```python
from build123d import *

# Parameters (mm, degrees)
SKETCH1_R           = 10.75
SKETCH1_R_2         = 5.25
BOSS_EXTRUDE1_DEPTH = 5
CHAMFER1_SIZE       = 0.5


with BuildPart() as part:
    # Sketch1 → Boss-Extrude1 (new body)
    with BuildSketch(Plane.XY):
        Circle(SKETCH1_R)
        Circle(SKETCH1_R_2, mode=Mode.SUBTRACT)
    extrude(amount=BOSS_EXTRUDE1_DEPTH)

    # Chamfer1
    chamfer1_edges = [part.edges().sort_by_distance(p)[0] for p in [
        (-10.75, 0, 0),
        (-10.75, 0, 5),
        (-5.25, 0, 0),
        (-5.25, 0, 5),
    ]]
    chamfer(chamfer1_edges, length=CHAMFER1_SIZE)


solid = part.part
```
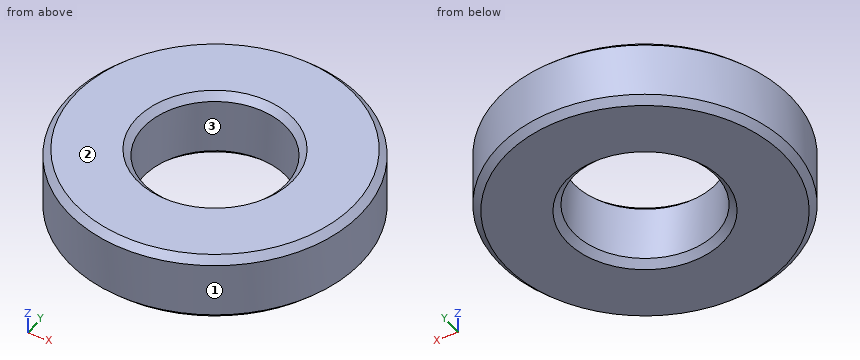
Input: part model. Units: mm. Frame: model coordinates. Face numbers are marked on the shaded views. Give positions to 0.01 mm unless a question says otherwise; leave off trailing zeros. Loops run counter-clockwise (first coordinate to the right, second up) from the corner with the lowest first, then second, coordinate; pieces in that order, holes last.
1) Contact query for flat-ended pins moving along their axis: pin 1 (3 mm diameter, centred on x = -7.5, z = 3.5, fed in from -Y); pin 2 (1.5 mm diameter, centred on y = -7.5, z = 3.5, fed in from +X); pin 3 (1.5 mm diameter, centred on x = -6.5, y = 8.5, fed in from +Z); pin 4 (8.5 mm diameter, centred on x = 0, y = 0, fed in from +Z). Output: stop coordinate, or through.
A:
pin 1: stops at y = -8.92
pin 2: stops at x = 8.37
pin 3: stops at z = 5
pin 4: passes through
2) Section query C-C on z = 4.75. Return the cut outline in (x, y).
A:
outline: circle Ø21 at (0, 0); hole circle Ø11 at (0, 0)
3) Section query A-A on y = 0. Return the cut outline in (x, z), and give its area (3 significant figures).
A:
outline: (-10.75, 0.5) - (-10.25, 0) - (-5.75, 0) - (-5.25, 0.5) - (-5.25, 4.5) - (-5.75, 5) - (-10.25, 5) - (-10.75, 4.5) - close; (5.25, 0.5) - (5.75, 0) - (10.25, 0) - (10.75, 0.5) - (10.75, 4.5) - (10.25, 5) - (5.75, 5) - (5.25, 4.5) - close
area: 54.0 mm2
4) Line query: L1, parallel to Y at x = 0, z = 3; L2, parallel to X at y = 1.75, z = 4.15; L3, parallel to X at y = -1, z = 2.8. Output: solid intervals per line, ascending.
A:
L1: y = -10.75 to -5.25, 5.25 to 10.75
L2: x = -10.61 to -4.95, 4.95 to 10.61
L3: x = -10.7 to -5.15, 5.15 to 10.7
5) Section query D-D on z = 3. Return the cut outline in (x, y).
A:
outline: circle Ø21.5 at (0, 0); hole circle Ø10.5 at (0, 0)
6) Mould query, pull axis Y, two halves, no side actions, for the marked faces 1, 2 and 3. Classes: released by +Y, released by -Y, zero draft, split by the parting line, or undercut.
A:
face 1: split by the parting line
face 2: zero draft
face 3: undercut
